Check sheet for the modelled part. Datum: model origin and axes. Units: mm. Face numbers are marked on the shaded views. Round coordinates to 2 decimals unless told otherwise and drop trailing zeros. Write each loop counter-clockwise with the first axis right and the second up, starting at its lowest first coordinate (ties: lowest second). Pieces come first, ordered by that corner, then holes.
Item 1: Depth check by flat-ended pin: pin 1 (3 mm diameter, centred on x = -113, y = -8.5, fed in from +Z). Enter the tip coordinate at first touch or a pass-through.
Item 2: Release check for a two-part mould opening along X. For the marked faces 1 and 2 record: pulls with the +X half, pulls with the -X half, needs draft (parallel to the pull), parting line crosses it, or undercut.
Item 3: Material ranges on line 1 along X through (y, z) = (15, 13); line 2 along Z through (x, y) = (-301, -56), recorded low to high.
Item 4: Section check B-B, the plane y = -1. Record the cut outline in (x, z).
Item 5: Section check C-C, the plane x = -397.5. Record the cut outline in (y, z).
Item 6: Section check A-A, the plane z = 10.5. Record the cut outline in (x, y).
from build123d import *

# Parameters (mm, degrees)
SKETCH_1_W      = 1518
SKETCH_1_H      = 200
EXTRUDE_1_DEPTH = 1
SKETCH_2_W      = 3
SKETCH_2_H      = 200
EXTRUDE_2_DEPTH = 40


with BuildPart() as part:
    # 草图1 → 凸台-拉伸1 (new body)
    with BuildSketch(Plane.XY):
        Rectangle(SKETCH_1_W, SKETCH_1_H)
    extrude(amount=EXTRUDE_1_DEPTH)

    # 草图2 → 凸台-拉伸2 (add)
    with BuildSketch(Plane.XY.offset(1)):
        with Locations((-757.5, 0)):
            Rectangle(SKETCH_2_W, SKETCH_2_H)
    extrude_2 = extrude(amount=EXTRUDE_2_DEPTH)

    # 镜向1: 凸台-拉伸2 across plane
    add(extrude_2.mirror(Plane(origin=(0, 0, 0), x_dir=(0, 0, 1), z_dir=(1, 0, 0))))


solid = part.part
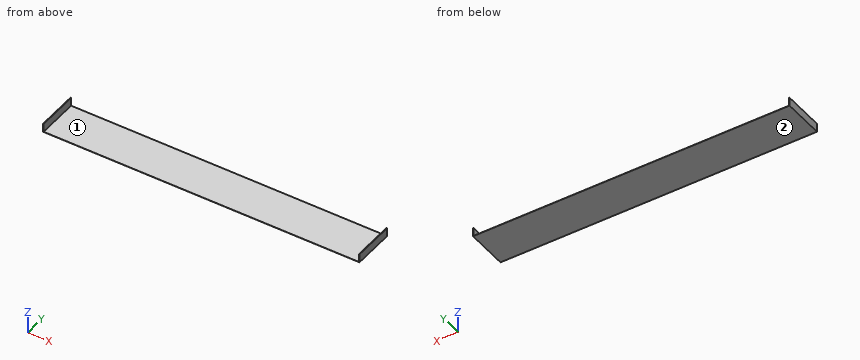
Values found:
1. pin 1: stops at z = 1
2. face 1: undercut
2. face 2: needs draft
3. line 1: x = -759 to -756, 756 to 759
3. line 2: z = 0 to 1
4. outline: (-759, 0) - (759, 0) - (759, 41) - (756, 41) - (756, 1) - (-756, 1) - (-756, 41) - (-759, 41) - close
5. outline: (-100, 0) - (100, 0) - (100, 1) - (-100, 1) - close
6. outline: (-759, -100) - (-756, -100) - (-756, 100) - (-759, 100) - close; (756, -100) - (759, -100) - (759, 100) - (756, 100) - close
